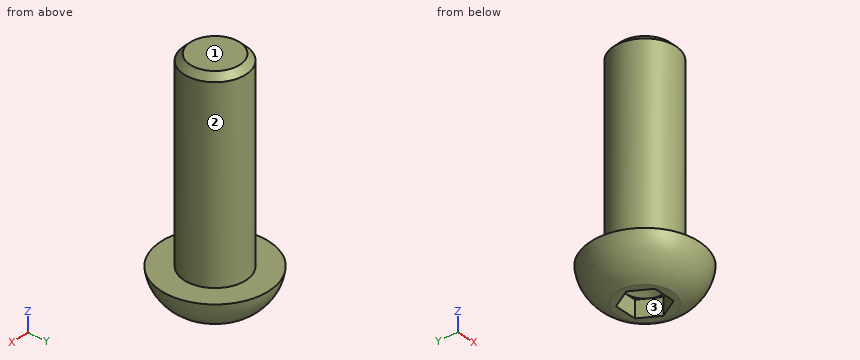
```python
from build123d import *

# Parameters (mm, degrees)
SKETCH_1_R          = 7
EXTRUDE_1_DEPTH     = 4.4
SKETCH_2_R          = 4
EXTRUDE_2_DEPTH     = 25
CHAMFER_1_SIZE      = 0.8
CUT_EXTRUDE_1_DEPTH = 2.2


with BuildPart() as part:
    # 草图1 → 凸台-拉伸1 (new body)
    with BuildSketch(Plane.XY):
        Circle(SKETCH_1_R)
    extrude(amount=-EXTRUDE_1_DEPTH)

    # 草图2 → 凸台-拉伸2 (add)
    with BuildSketch(Plane(origin=(0, 0, 0), x_dir=(-1, 0, 0), z_dir=(0, 0, -1))):
        Circle(SKETCH_2_R)
    extrude(amount=-EXTRUDE_2_DEPTH)

    # 倒角1
    chamfer_1_edges = [part.edges().sort_by_distance(p)[0] for p in [
        (4, 0, 25),
    ]]
    chamfer(chamfer_1_edges, length=CHAMFER_1_SIZE)

    # 草图3 → 切除-拉伸1 (cut)
    with BuildSketch(Plane.XY.offset(-4.4)):
        Polygon((1.443375673, 2.5), (-1.443375673, 2.5), (-2.886751346, 0), (-1.443375673, -2.5), (1.443375673, -2.5), (2.886751346, 0), align=None)
    extrude(amount=CUT_EXTRUDE_1_DEPTH, mode=Mode.SUBTRACT)

    # 草图4 → 切除-旋转1 (revolve, cut)
    with BuildSketch(Plane(origin=(0, 0, 0), x_dir=(0, 1, 0), z_dir=(-1, 0, 0)), mode=Mode.PRIVATE) as cut_revolve_1_sk:
        Polygon((0, 0.756624327), (-2.5, 2.2), (0, 2.2), align=None)
    revolve(cut_revolve_1_sk.sketch.rotate(Axis((0, 0, 0), (0, 0, 1)), 270), axis=Axis((0, 0, 0), (0, 0, 1)), mode=Mode.SUBTRACT)

    # 草图5 → 切除-旋转2 (revolve, cut)
    with BuildSketch(Plane(origin=(0, 0, 0), x_dir=(1, 0, 0), z_dir=(0, 1, 0))):
        with BuildLine():
            Line((-7, 0), (-7, 4.4))
            Line((-7, 4.4), (-3.5, 4.4))
            ThreePointArc((-3.5, 4.4), (-5.867796506, 2.691429039), (-7, 0))
        make_face()
    revolve(axis=Axis((0, 0, 0), (0, 0, 1)), mode=Mode.SUBTRACT)


solid = part.part
```
Geometry check sheet. Reference: the model listing, model coordinates, mm. Face numbers are marked on the shaded views. A direction names the side the tool comes from. Coordinates: 2 decimals unless noted, no trailing zeros. Loops run counter-clockwise (first coordinate to the right, second up) from the corner with the lowest first, then second, coordinate; pieces in that order, holes last.
Item 1: Go/stop test with flat-tipped pins: pin 1 Ø2 at (x, y) = (-3, -4.5) entering from +Z; pin 2 Ø3 at (y, z) = (3, 1) entering from -X; pin 3 Ø2 at (x, z) = (0.5, 14) entering from -Y. Record where each tip stops, or that it passes through.
Item 2: Thickness scan on line 1 (X direction, y = 0.25, z = 8.5); line 2 (Z direction, x = 5.5, y = -1.5); line 3 (Y direction, x = -3.25, z = 19.75). Record the ranges inside material, lowest first.
Item 3: Sectioned sample at A-A, the plane z = 19.75. Record the boundary of the cut face in (x, y), then the cut area to 3 significant figures.
Item 4: Access from +Z, -Z, +X, -X, +Y, -Y to the whole of each face (thin tool, end or side, straight path). Record for the marked faces 1, 2 and 3.
Check result:
1. pin 1: stops at z = 0
1. pin 2: stops at x = -6.74
1. pin 3: stops at y = -4
2. line 1: x = -3.99 to 3.99
2. line 2: z = -2.89 to 0
2. line 3: y = -2.33 to 2.33
3. outline: circle Ø8 at (0, 0)
3. area: 50.3 mm2
4. face 1: +Z, +X, -X, +Y, -Y
4. face 2: +Z
4. face 3: -Z
